from build123d import *

# Parameters (mm, degrees)
EXTRUDE_1_DEPTH     = 10
SKETCH_2_R          = 3.2
CUT_EXTRUDE_1_DEPTH = 25


with BuildPart() as part:
    # 草图1 → 凸台-拉伸1 (new, symmetric)
    with BuildSketch(Plane.XY):
        with BuildLine():
            Line((-140, 15), (140, 15))
            ThreePointArc((140, 15), (155, 0), (140, -15))
            Line((140, -15), (-140, -15))
            ThreePointArc((-140, -15), (-155, 0), (-140, 15))
        make_face()
    extrude(amount=EXTRUDE_1_DEPTH, both=True)

    # 草图2 → 切除-拉伸1 (cut, symmetric)
    with BuildSketch(Plane.XY):
        with Locations(Location((-140, 0, 0), (0, 0, 180))):
            Circle(SKETCH_2_R)
        with Locations(Location((140, 0, 0), (0, 0, 180))):
            Circle(SKETCH_2_R)
    extrude(amount=CUT_EXTRUDE_1_DEPTH, both=True, mode=Mode.SUBTRACT)


solid = part.part
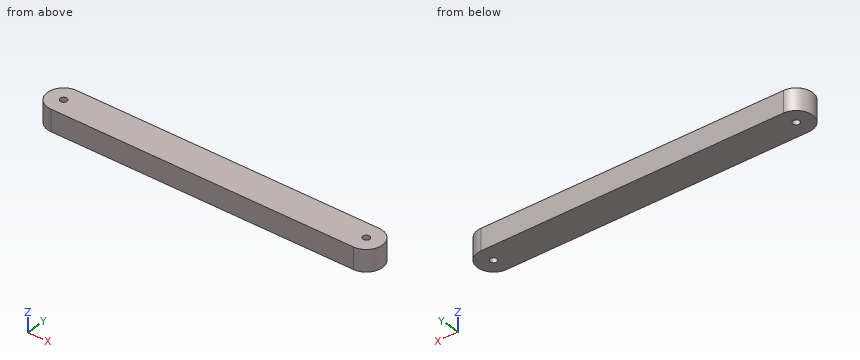
Geometry: final body of the model. Coordinates: model frame, mm. Round coordinates to 2 decimals unless told otherwise and drop trailing zeros. Loops run counter-clockwise (first coordinate to the right, second up) from the corner with the lowest first, then second, coordinate; pieces in that order, holes last. Notation, with made-up numbers: M -18.75,79.25 L 23.25,79.25 A31 cw 23.25,104.25 Z; hole C -18,-5 d5. An arc over 180 degrees is marked long. Put each result on its own line as item: value. Start each with the question number.
(1) Contact query for flat-ended pins moving along their axis: pin 1 Ø5 at (x, y) = (-140, 0) entering from -Z; pin 2 Ø5 at (y, z) = (-8.5, -1) entering from +X; pin 3 Ø1.5 at (y, z) = (-9, -8) entering from -X. Output: stop coordinate, or through.
(2) Material intervals for line 1 along Y through (x, z) = (140, -4.5); line 2 along X through (y, z) = (-11, -3.75); line 3 along X through (y, z) = (-4, 5.25), sorted ascending. Write a range as [from, to].
(3) Section query A-A (y = 0). Return loops of the section in (x, z).
(4) Section query B-B (z = -2.75). Return loops of the section in (x, y), then the cut area to 3 significant figures.
Findings below:
1. pin 1: passes through
1. pin 2: stops at x = 153.75
1. pin 3: stops at x = -152.53
2. line 1: y = [-15, -3.2], [3.2, 15]
2. line 2: x = [-150.2, 150.2]
2. line 3: x = [-154.46, 154.46]
3. outline: M -155,-10 L -143.2,-10 L -143.2,10 L -155,10 Z; M -136.8,-10 L 136.8,-10 L 136.8,10 L -136.8,10 Z; M 143.2,-10 L 155,-10 L 155,10 L 143.2,10 Z
4. outline: M -140,-15 L 140,-15 A15 ccw 140,15 L -140,15 A15 ccw Z; hole C -140,0 d6.4; hole C 140,0 d6.4
4. area: 9,040 mm2
